from build123d import *

# Parameters (mm, degrees)
SKETCH1_W                  = 95
SKETCH1_H                  = 223.5
BOSS_EXTRUDE1_DEPTH        = 15
CUT_EXTRUDE1_DEPTH         = 123.349141803
M6_CLEARANCE_HOLE1_D       = 6.6
M6_CLEARANCE_HOLE1_DEPTH   = 19.75
M6_CLEARANCE_HOLE1_TIP     = 1.982840043
M6_TAPPED_HOLE1_D          = 5
M6_TAPPED_HOLE1_DEPTH      = 15
M6_TAPPED_HOLE1_TIP        = 1.502151548
F_5_0MM_BLIND_HOLE_1_D     = 5
F_5_0MM_BLIND_HOLE_1_DEPTH = 8
F_5_0MM_BLIND_HOLE_1_TIP   = 1.502151548
F_5_0MM_BLIND_HOLE_2_D     = 5
F_5_0MM_BLIND_HOLE_2_DEPTH = 8
F_5_0MM_BLIND_HOLE_2_TIP   = 1.502151548
M5_TAPPED_HOLE1_D          = 4.2
M5_TAPPED_HOLE1_DEPTH      = 12.4
M5_TAPPED_HOLE1_TIP        = 1.2618073


with BuildPart() as part:
    # Sketch1 → Boss-Extrude1 (new body)
    with BuildSketch(Plane(origin=(0, 0, 0), x_dir=(0, 0, -1), z_dir=(1, 0, 0))):
        Rectangle(SKETCH1_W, SKETCH1_H)
    extrude(amount=BOSS_EXTRUDE1_DEPTH)

    # Sketch2 → Cut-Extrude1 (cut, through all)
    with BuildSketch(Plane.ZY):
        with BuildLine():
            Line((22.5, -61.75), (2.5, -61.75))
            ThreePointArc((2.5, -61.75), (-1.035533906, -63.214466094), (-2.5, -66.75))
            Line((-2.5, -66.75), (-2.5, -111.75))
            Line((-2.5, -111.75), (27.5, -111.75))
            Line((27.5, -111.75), (27.5, -66.75))
            ThreePointArc((27.5, -66.75), (26.035533906, -63.214466094), (22.5, -61.75))
        make_face()
        with BuildLine():
            Line((-27.5, 19.75), (27.5, 19.75))
            ThreePointArc((27.5, 19.75), (31.035533906, 21.214466094), (32.5, 24.75))
            Line((32.5, 24.75), (32.5, 94.75))
            ThreePointArc((32.5, 94.75), (31.035533906, 98.285533906), (27.5, 99.75))
            Line((27.5, 99.75), (-27.5, 99.75))
            ThreePointArc((-27.5, 99.75), (-31.035533906, 98.285533906), (-32.5, 94.75))
            Line((-32.5, 94.75), (-32.5, 24.75))
            ThreePointArc((-32.5, 24.75), (-31.035533906, 21.214466094), (-27.5, 19.75))
        make_face()
    extrude(amount=-CUT_EXTRUDE1_DEPTH, mode=Mode.SUBTRACT)

    # M6 Clearance Hole1
    with Locations(Plane(origin=(0, 111.75, 0), x_dir=(1, 0, 0), z_dir=(0, 1, 0))):
        with Locations((7.5, -20), (7.5, 20)):
            Hole(M6_CLEARANCE_HOLE1_D / 2, depth=M6_CLEARANCE_HOLE1_DEPTH)
            with Locations((0, 0, -(M6_CLEARANCE_HOLE1_DEPTH + M6_CLEARANCE_HOLE1_TIP / 2))):  # 118° drill point
                Cone(0, M6_CLEARANCE_HOLE1_D / 2, M6_CLEARANCE_HOLE1_TIP, mode=Mode.SUBTRACT)

    # M6 Tapped Hole1
    with Locations(Plane(origin=(0, -111.75, 0), x_dir=(-1, 0, 0), z_dir=(0, -1, 0))):
        with Locations((-7.5, -40), (-7.5, 40)):
            Hole(M6_TAPPED_HOLE1_D / 2, depth=M6_TAPPED_HOLE1_DEPTH)
            with Locations((0, 0, -(M6_TAPPED_HOLE1_DEPTH + M6_TAPPED_HOLE1_TIP / 2))):  # 118° drill point
                Cone(0, M6_TAPPED_HOLE1_D / 2, M6_TAPPED_HOLE1_TIP, mode=Mode.SUBTRACT)

    # Ø5.0mm blind hole 1
    with Locations(Plane(origin=(0, -111.75, 0), x_dir=(-1, 0, 0), z_dir=(0, -1, 0))):
        with Locations((-7.5, 10)):
            Hole(F_5_0MM_BLIND_HOLE_1_D / 2, depth=F_5_0MM_BLIND_HOLE_1_DEPTH)
            with Locations((0, 0, -(F_5_0MM_BLIND_HOLE_1_DEPTH + F_5_0MM_BLIND_HOLE_1_TIP / 2))):  # 118° drill point
                Cone(0, F_5_0MM_BLIND_HOLE_1_D / 2, F_5_0MM_BLIND_HOLE_1_TIP, mode=Mode.SUBTRACT)

    # Ø5.0mm blind hole 2
    with Locations(Plane(origin=(0, 111.75, 0), x_dir=(1, 0, 0), z_dir=(0, 1, 0))):
        with Locations((7.5, -40), (7.5, 40)):
            Hole(F_5_0MM_BLIND_HOLE_2_D / 2, depth=F_5_0MM_BLIND_HOLE_2_DEPTH)
            with Locations((0, 0, -(F_5_0MM_BLIND_HOLE_2_DEPTH + F_5_0MM_BLIND_HOLE_2_TIP / 2))):  # 118° drill point
                Cone(0, F_5_0MM_BLIND_HOLE_2_D / 2, F_5_0MM_BLIND_HOLE_2_TIP, mode=Mode.SUBTRACT)

    # M5 Tapped Hole1
    with Locations(Plane(origin=(15, 0, 0), x_dir=(0, 0, -1), z_dir=(1, 0, 0))):
        with Locations((40, 66.75), (-40, 66.75), (40, -78.25), (-40, -78.25)):
            Hole(M5_TAPPED_HOLE1_D / 2, depth=M5_TAPPED_HOLE1_DEPTH)
            with Locations((0, 0, -(M5_TAPPED_HOLE1_DEPTH + M5_TAPPED_HOLE1_TIP / 2))):  # 118° drill point
                Cone(0, M5_TAPPED_HOLE1_D / 2, M5_TAPPED_HOLE1_TIP, mode=Mode.SUBTRACT)


solid = part.part
Read the model definition and answer for the solid it produces. Units are mm, in the model's axes. A direction names the side the tool comes from. Round coordinates to 2 decimals unless told otherwise and drop trailing zeros. Write each loop counter-clockwise with the first axis right and the second up, starting at its lowest first coordinate (ties: lowest second). Pieces come first, ordered by that corner, then holes.
1. Determine the mould class of faces 6 (the face through (1.56, -78.61, 40.08)), 7 (the face through (7, 60, -32.5)), 8 (the face through (6.96, -104.14, 42.44)) for opening direction X: pulls with the +X half, pulls with the -X half, needs draft (parallel to the pull), parting line crosses it, or undercut.
2. Which of the six approach directions +Z, -Z, +X, -X, +Y, -Y give full straight-line access (tool end or side, diameter ignored) to faces 1 (the face through (7.4, 98.25, 31.07)), 2 (the face through (9, -108, -8)), 3 (the face through (8.713, -79.528, -41.666)), 4 (the face through (7, -89, -2.5)), 5 (the face through (7.44, 102.51, 39.57))?
3. Given pin 1 Ø4 at (x, z) = (7.5, -10) entering from -Y; pin 2 Ø5.5 at (x, z) = (7.5, 20) entering from -Y, each flat-ended and moving along its own axis, determine where each tip first touches the part or whether it passes through.
4. The part is cut by section C-C, the plane z = 25.5. Determine the outline of the cut face in (x, y).
5. The part is cut by section B-B, the plane y = -85.5. Determine the outline of the cut face in (x, z), then the cut area to 3 significant figures.
6. The part is cut by section A-A, the plane z = -20. Determine the outline of the cut face in (x, y).
7. Straight lines are drawn through the part: L1, parallel to Y at x = 11, z = 40; L2, parallel to Z at x = 7.75, y = -78.25; L3, parallel to Y at x = 3.75, z = -20. For each, find the intervals that lie inside material, in ascending order.
Values:
1. face 6: pulls with the +X half
1. face 7: needs draft
1. face 8: undercut
2. face 1: +X, -X
2. face 2: -Y
2. face 3: +X
2. face 4: +X, -X, -Y
2. face 5: +Y
3. pin 1: stops at y = -103.45
3. pin 2: stops at y = -61.76
4. outline: (0, -62.75) - (15, -62.75) - (15, 19.75) - (0, 19.75) - close; (0, 99.75) - (15, 99.75) - (15, 111.75) - (0, 111.75) - close
5. outline: (0, -47.5) - (15, -47.5) - (15, -2.5) - (0, -2.5) - close; (0, 27.5) - (15, 27.5) - (15, 47.5) - (0, 47.5) - close
5. area: 975 mm2
6. outline: (0, -111.75) - (15, -111.75) - (15, 19.75) - (0, 19.75) - close; (0, 99.75) - (4.2, 99.75) - (4.2, 111.75) - (0, 111.75) - close; (10.8, 99.75) - (15, 99.75) - (15, 111.75) - (10.8, 111.75) - close
7. L1: y = -111.75 to -80.35, -76.15 to 64.65, 68.85 to 111.75
7. L2: z = -47.5 to -42.1, -37.9 to -2.5, 27.5 to 37.9, 42.1 to 47.5
7. L3: y = -111.75 to 19.75, 99.75 to 111.75
